from build123d import *

# Parameters (mm, degrees)
SKETCH1_R           = 55
SKETCH1_R_2         = 27.5
BOSS_EXTRUDE1_DEPTH = 20
CHAMFER1_SIZE       = 2


with BuildPart() as part:
    # Sketch1 → Boss-Extrude1 (new body)
    with BuildSketch(Plane.XY):
        Circle(SKETCH1_R)
        Circle(SKETCH1_R_2, mode=Mode.SUBTRACT)
    extrude(amount=BOSS_EXTRUDE1_DEPTH)

    # Chamfer1
    chamfer1_edges = [part.edges().sort_by_distance(p)[0] for p in [
        (-55, 0, 20),
        (-27.5, 0, 0),
        (-27.5, 0, 20),
    ]]
    chamfer(chamfer1_edges, length=CHAMFER1_SIZE)


solid = part.part
The model under review builds one solid part; all positions refer to its coordinate system, in mm. Give positions to 0.01 mm unless a question says otherwise; leave off trailing zeros. Write each loop counter-clockwise with the first axis right and the second up, starting at its lowest first coordinate (ties: lowest second). Pieces come first, ordered by that corner, then holes.
1. Add section A-A, the plane x = 0. Write out the cut boundary in (y, z), plus the area to 3 significant figures.
2. Add section C-C, the plane z = 16.5. Write out the cut boundary in (x, y).
3. Wall thickness on L1, parallel to Y at x = 7, z = 6.5; L2, parallel to Y at x = -3.5, z = 9; L3, parallel to X at y = 20, z = 7.25: over which ranges is each line inside the solid? List them lowest first.
4. Draft analysis for pull direction Y (two halves, no side actions). For faces 1 (the flat face through (24, -24, 0)), 2 (the cylindrical face through (-11.923, -53.692, 8.874)), 3 (the cylindrical face through (-5.961, -26.846, 9.888)), state which applies: +Y half, -Y half, draft (parallel to the pull), parting line (faces both ways), or undercut.
5. For P1, Ø10, axis at x = 30.5, z = 4, coming from the +Y side; P2, Ø6, axis at x = 24, z = 12, coming from the -Y side; P3, Ø8, axis at x = 7.5, z = 17, coming from the -Y side, all flat-tipped, find the tip position at first contact; note any pin that passes through.
Worked answers:
1. outline: (-55, 0) - (-29.5, 0) - (-27.5, 2) - (-27.5, 18) - (-29.5, 20) - (-53, 20) - (-55, 18) - close; (27.5, 2) - (29.5, 0) - (55, 0) - (55, 18) - (53, 20) - (29.5, 20) - (27.5, 18) - close
1. area: 1,090 mm2
2. outline: circle Ø110 at (0, 0); hole circle Ø55 at (0, 0)
3. L1: y = -54.55 to -26.59, 26.59 to 54.55
3. L2: y = -54.89 to -27.28, 27.28 to 54.89
3. L3: x = -51.23 to -18.87, 18.87 to 51.23
4. face 1: draft
4. face 2: parting line
4. face 3: undercut
5. P1: stops at y = 48.73
5. P2: stops at y = -50.83
5. P3: stops at y = -54.89
